Build history of the part. All positions in model axes, mm. A direction names the side the tool comes from. Give positions to 0.01 mm unless a question says otherwise; leave off trailing zeros. Order: outer loops, then holes, each group sorted by start corner. A loop starts at its lowest first (then second) coordinate and runs counter-clockwise, first axis right, second up. Notation, with made-up numbers: M 27,77 L 63,77 A11 cw 63,98 Z; hole C -20,34 d5. An arc over 180 degrees is marked long. One line per item, written item: value.
from build123d import *

# Parameters (mm, degrees)
BASE_BLOCK_PROFILE_W        = 80
BASE_BLOCK_PROFILE_H        = 40
BASE_BLOCK_80X40X42_DEPTH   = 42
TOP_SLOT_PROFILE_W          = 34
TOP_SLOT_PROFILE_H          = 30
TOP_SLOT_CUT_10_DEPTH       = 10
GROOVE_CUT_22_DEPTH         = 22
GROOVE_INFILL_BOSS_10_DEPTH = 10
GROOVE_UNDERCUT_10_DEPTH    = 10
ROUNDED_END_CUT_DEPTH       = 42
ARCH_PROFILE_R              = 8
ARCH_CUT_10_DEPTH           = 10
SIDE_SLOT_PROFILE_W         = 22
SIDE_SLOT_PROFILE_H         = 40
SIDE_SLOT_CUT_8_DEPTH       = 8
INCLINED_SLOT_PROFILE_W     = 6
INCLINED_SLOT_PROFILE_H     = 10
INCLINED_SLOT_CUT_46_DEPTH  = 46
BORE_16_PROFILE_R           = 8
BORE_16_CUT_46_DEPTH        = 46


with BuildPart() as part:
    # Base Block Profile → Base Block 80x40x42 (new body)
    with BuildSketch(Plane.XY):
        with Locations((40, 20)):
            Rectangle(BASE_BLOCK_PROFILE_W, BASE_BLOCK_PROFILE_H)
    extrude(amount=-BASE_BLOCK_80X40X42_DEPTH)

    # Top Slot Profile → Top Slot Cut 10 (cut)
    with BuildSketch(Plane.XY):
        with Locations((63, 25)):
            Rectangle(TOP_SLOT_PROFILE_W, TOP_SLOT_PROFILE_H)
    extrude(amount=-TOP_SLOT_CUT_10_DEPTH, mode=Mode.SUBTRACT)

    # Groove Profile → Groove Cut 22 (cut)
    with BuildSketch(Plane.XY.offset(-10)):
        Polygon((46, 40), (80, 10), (80, 40), align=None)
    extrude(amount=-GROOVE_CUT_22_DEPTH, mode=Mode.SUBTRACT)

    # Groove Infill Profile → Groove Infill Boss 10 (add)
    with BuildSketch(Plane.XY):
        with BuildLine():
            Line((46, 40), (46, 10))
            Line((46, 10), (80, 10))
            ThreePointArc((80, 10), (68.671568098, 31.427777177), (46, 40))
        make_face()
    extrude(amount=-GROOVE_INFILL_BOSS_10_DEPTH)

    # Groove Undercut Profile → Groove Undercut 10 (cut)
    with BuildSketch(Plane.XY.offset(-32)):
        with BuildLine():
            Line((46, 40), (80, 40))
            Line((80, 40), (80, 10))
            ThreePointArc((80, 10), (68.671568098, 31.427777177), (46, 40))
        make_face()
    extrude(amount=-GROOVE_UNDERCUT_10_DEPTH, mode=Mode.SUBTRACT)

    # Rounded End Profile → Rounded End Cut (cut)
    with BuildSketch(Plane.XY):
        with BuildLine():
            ThreePointArc((45, 0), (30, 15), (15, 0))
            Line((15, 0), (30, 0))
            Line((30, 0), (45, 0))
        make_face()
    extrude(amount=-ROUNDED_END_CUT_DEPTH, mode=Mode.SUBTRACT)

    # Arch Profile → Arch Cut 10 (cut)
    with BuildSketch(Plane(origin=(0, 40, 0), x_dir=(1, 0, 0), z_dir=(0, 1, 0))):
        with Locations(Location((30, 21, 0), (0, 0, 270))):
            Circle(ARCH_PROFILE_R)
    extrude(amount=-ARCH_CUT_10_DEPTH, mode=Mode.SUBTRACT)

    # Side Slot Profile → Side Slot Cut 8 (cut)
    with BuildSketch(Plane.ZY):
        with Locations((-21, 20)):
            Rectangle(SIDE_SLOT_PROFILE_W, SIDE_SLOT_PROFILE_H)
    extrude(amount=-SIDE_SLOT_CUT_8_DEPTH, mode=Mode.SUBTRACT)

    # Inclined Slot Profile → Inclined Slot Cut 46 (cut)
    with BuildSketch(Plane.ZY.offset(-8)):
        with Locations((-21, 35)):
            Rectangle(INCLINED_SLOT_PROFILE_W, INCLINED_SLOT_PROFILE_H)
    extrude(amount=-INCLINED_SLOT_CUT_46_DEPTH, mode=Mode.SUBTRACT)

    # Bore Ø16 Profile → Bore Ø16 Cut 46 (cut)
    with BuildSketch(Plane(origin=(0, 30, 0), x_dir=(1, 0, 0), z_dir=(0, 1, 0))):
        with Locations(Location((30, 21, 0), (0, 0, 270))):
            Circle(BORE_16_PROFILE_R)
    extrude(amount=-BORE_16_CUT_46_DEPTH, mode=Mode.SUBTRACT)


solid = part.part
1) Tool access for faces 5 (the face through (8, 20, -21)), 6 (the face through (0, 20, -5)), 7 (the face through (15, 30, -21)), 8 (the face through (35.27, 26.54, -14.98)), 9 (the face through (65, 27, -10)): list every direction of +Z, -Z, +X, -X, +Y, -Y with a clear straight run to the whole face (end or side of a thin tool).
Check values:
face 5: -X, +Y, -Y
face 6: +Z, -Z, -X, +Y, -Y
face 7: -X, +Y
face 8: +Y, -Y
face 9: +X, +Y
2) Mould opens along Z. For faces 1 (the face through (39, 20, -42)), 2 (the face through (80, 5, -21)), 3 (the face through (39, 20, 0)), 4 (the face through (4, 20, -32)) say: released by +Z, released by -Z, zero draft, split by the parting line, or undercut.
Check values:
face 1: released by -Z
face 2: zero draft
face 3: released by +Z
face 4: undercut
3) Drill centre lines: probe 1 along Z at (x, y) = (30, 24); probe 2 along Z at (x, y) = (53, 37.5); probe 3 along X at (y, z) = (29, -19.5). Where is each one in solid material? Low to high. Write a range as from..to.
Check values:
probe 1: -42..-29, -13..0
probe 2: -42..-32, -10..0
probe 3: 8..22.14, 37.86..58.47
4) Saw through at C-C, the plane y = 20.5. Write the cut outline in (x, z), then the cut area to 3 significant figures.
Check values:
outline: M 0,-42 L 76.92,-42 L 76.92,-32 L 68.1,-32 L 68.1,-10 L 76.92,-10 L 76.92,0 L 0,0 L 0,-10 L 8,-10 L 8,-32 L 0,-32 Z; hole C 30,-21 d16
area: 2,660 mm^2
5) Saw through at A-A, the plane x = 30. Write the cut outline in (y, z), then the cut area to 3 significant figures.
Check values:
outline: M 15,-42 L 40,-42 L 40,-29 L 15,-29 Z; M 15,-13 L 40,-13 L 40,0 L 15,0 Z
area: 650 mm^2
6) Saw through at D-D, the plane y = 5. Write the cut outline in (x, z).
Check values:
outline: M 0,-42 L 15.86,-42 L 15.86,0 L 0,0 L 0,-10 L 8,-10 L 8,-32 L 0,-32 Z; M 44.14,-42 L 80,-42 L 80,0 L 44.14,0 Z
7) Saw through at B-B, the plane z = -21. Write the cut outline in (x, y), then the cut area to 3 significant figures.
Check values:
outline: M 8,0 L 15,0 A15 cw 22,12.69 L 22,30 L 8,30 Z; M 38,12.69 A15 cw 45,0 L 80,0 L 80,10 L 54,32.94 L 54,30 L 38,30 Z
area: 1,330 mm^2
8) Pin check, flat tips, straight feed: pin 1 (0.9 mm diameter, centred on y = 31, z = -22.5, fed in from -X); pin 2 (2 mm diameter, centred on y = 13, z = -12, fed in from -X); pin 3 (1.8 mm diameter, centred on x = 45.5, z = -22, fed in from +Y). Stop position of each tip, or through.
Check values:
pin 1: x = 54
pin 2: x = 8
pin 3: y = 30
